Here's the drawing with two shaded views (mm, measured from the low corner). I have some questions. Round coordinates to 2 decimals unless told otherwise and drop trailing zeros. Loops run counter-clockwise (first coordinate to the right, second up) from the corner with the lowest first, then second, coordinate; pieces in that order, holes last.
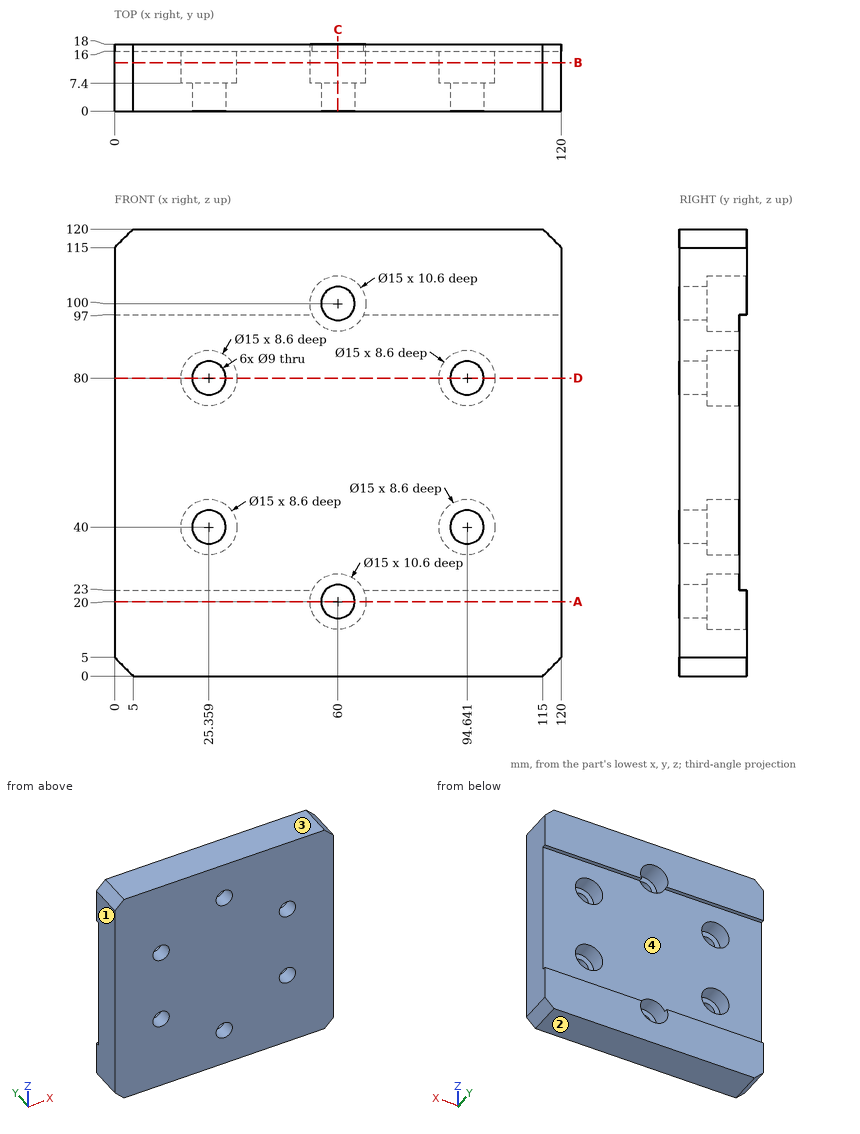
Item 1: If we section it at A-A, the plane z = 20: Please give me the cut outline in (x, y).
Results list:
outline: (0, 0) - (55.5, 0) - (55.5, 7.4) - (52.5, 7.4) - (52.5, 18) - (0, 18) - close; (64.5, 0) - (120, 0) - (120, 18) - (67.5, 18) - (67.5, 7.4) - (64.5, 7.4) - close
Item 2: We'd pull the mould along Z, two halves only. Please class the marked faces 1, 2, 3 and 4: released by +Z, released by -Z, zero draft, split by the parting line, or undercut.
Results list:
face 1: zero draft
face 2: released by -Z
face 3: released by +Z
face 4: undercut
Item 3: If we section it at D-D, the plane z = 80: Please give me the cut outline in (x, y), then the cut area to 3 significant figures.
Results list:
outline: (0, 0) - (20.86, 0) - (20.86, 7.4) - (17.86, 7.4) - (17.86, 16) - (0, 16) - close; (29.86, 0) - (90.14, 0) - (90.14, 7.4) - (87.14, 7.4) - (87.14, 16) - (32.86, 16) - (32.86, 7.4) - (29.86, 7.4) - close; (99.14, 0) - (120, 0) - (120, 16) - (102.14, 16) - (102.14, 7.4) - (99.14, 7.4) - close
area: 1,530 mm2
Item 4: If we section it at B-B, the plane y = 13: Please give me the cut outline in (x, z), then the cut area to 3 significant figures.
Results list:
outline: (0, 5) - (5, 0) - (115, 0) - (120, 5) - (120, 115) - (115, 120) - (5, 120) - (0, 115) - close; hole circle Ø15 at (25.36, 40); hole circle Ø15 at (25.36, 80); hole circle Ø15 at (60, 20); hole circle Ø15 at (60, 100); hole circle Ø15 at (94.64, 40); hole circle Ø15 at (94.64, 80)
area: 13,300 mm2
Item 5: If I drill on line 1 along X through (y, z) = (12, 40); line 2 along Z through (x, y) = (27, 5.25); line 3 along X through (y, z) = (5.25, 40), over which ranges is the centre line in solid material (lowest first)?
Results list:
line 1: x = 0 to 17.86, 32.86 to 87.14, 102.14 to 120
line 2: z = 0 to 35.81, 44.19 to 75.81, 84.19 to 120
line 3: x = 0 to 20.86, 29.86 to 90.14, 99.14 to 120
Item 6: Will these pins go through, and if not, where does the flat tip stop? pin 1 (12 mm diameter, centred on x = 25.36, z = 40, fed in from +Y); pin 2 (16.5 mm diameter, centred on x = 28, z = 41.5, fed in from +Y).
Results list:
pin 1: stops at y = 7.4
pin 2: stops at y = 16
Item 7: If we section it at C-C, the plane x = 60: Please give me the cut outline in (y, z).
Results list:
outline: (0, 0) - (18, 0) - (18, 12.5) - (7.4, 12.5) - (7.4, 15.5) - (0, 15.5) - close; (0, 24.5) - (7.4, 24.5) - (7.4, 27.5) - (16, 27.5) - (16, 92.5) - (7.4, 92.5) - (7.4, 95.5) - (0, 95.5) - close; (0, 104.5) - (7.4, 104.5) - (7.4, 107.5) - (18, 107.5) - (18, 120) - (0, 120) - close
